Source: CAD feature listing. Evaluate the final solid. Frame: model axes, mm. A direction names the side the tool comes from. Give positions to 0.01 mm unless a question says otherwise; leave off trailing zeros. Order: outer loops, then holes, each group sorted by start corner. A loop starts at its lowest first (then second) coordinate and runs counter-clockwise, first axis right, second up. Notation, with made-up numbers: M -28,-38.5 L -15,-38.5 A28 cw -15,-17.5 Z; hole C 74.25,-3.75 d1. An arc over 180 degrees is marked long. Return JSON: item names as keys, results as strings.
from build123d import *

# Parameters (mm, degrees)
CHAMFER1_SIZE = 0.5


with BuildPart() as part:
    # Sketch1 → Revolve1 (revolve)
    with BuildSketch(Plane.XY, mode=Mode.PRIVATE) as revolve1_sk:
        Polygon((1009, 204.198665167), (1009, 219.898665167), (1006.5, 219.898665167), (1006.5, 222.898665167), (1016.5, 222.898665167), (1016.5, 204.198665167), align=None)
    revolve(revolve1_sk.sketch.rotate(Axis((1016.5, 222.898665167, 0), (0, -1, 0)), 270), axis=Axis((1016.5, 222.898665167, 0), (0, -1, 0)))

    # Chamfer1
    chamfer1_edges = [part.edges().sort_by_distance(p)[0] for p in [
        (1016.5, 222.898665167, -10),
        (1016.5, 219.898665167, -10),
        (1016.5, 204.198665167, -7.5),
    ]]
    chamfer(chamfer1_edges, length=CHAMFER1_SIZE)


solid = part.part
1. Section query D-D (y = 221.25). Return loops of the section in (x, z), then the cut area to 3 significant figures.
Evaluation:
{"outline": "C 1016.5,0 d20", "area": "314 mm^2"}
2. Ray query, probe 1 along Y at (x, z) = (1022.75, -6); probe 2 along X at (y, z) = (212.5, 0.25); probe 3 along Z at (x, y) = (1013, 219.5). Return the intervals inside material, ascending.
Evaluation:
{"probe 1": "y = 219.9 to 222.9", "probe 2": "x = 1009 to 1024", "probe 3": "z = -6.63 to 6.63"}
3. Section query B-B (x = 1016.5). Return loops of the section in (y, z), then the cut area to 3 significant figures.
Evaluation:
{"outline": "M 204.2,-7 L 204.7,-7.5 L 219.9,-7.5 L 219.9,-9.5 L 220.4,-10 L 222.4,-10 L 222.9,-9.5 L 222.9,9.5 L 222.4,10 L 220.4,10 L 219.9,9.5 L 219.9,7.5 L 204.7,7.5 L 204.2,7 Z", "area": "295 mm^2"}
4. First-contact query: pin 1 (1 mm diameter, centred on x = 1020.5, y = 207, fed in from -Z); pin 2 (3 mm diameter, centred on x = 1009, y = 215.5, fed in from +Z); pin 3 (2 mm diameter, centred on x = 1010.5, y = 213, fed in from +Z). Flat tips, straight axial feed; report the tip coordinate or a pass-through.
Evaluation:
{"pin 1": "stops at z = -6.63", "pin 2": "stops at z = 4.5", "pin 3": "stops at z = 5.59"}
5. Section query C-C (y = 214). Return loops of the section in (x, z), then the cut area to 3 significant figures.
Evaluation:
{"outline": "C 1016.5,0 d15", "area": "177 mm^2"}
6. Section query A-A (z = 0). Return loops of the section in (x, y).
Evaluation:
{"outline": "M 1006.5,220.4 L 1007,219.9 L 1009,219.9 L 1009,204.7 L 1009.5,204.2 L 1023.5,204.2 L 1024,204.7 L 1024,219.9 L 1026,219.9 L 1026.5,220.4 L 1026.5,222.4 L 1026,222.9 L 1007,222.9 L 1006.5,222.4 Z"}
7. Set-up query: faces 1 (the face through (1016, 222.899, 0)), 2 (the face through (1008.7, 219.899, -0.7)). Return all of +Z, -Z, +X, -X, +Y, -Y with unobstructed straight access to the full face (end or side cutting, diameter ignored); none if empty.
Evaluation:
{"face 1": "+Z, -Z, +X, -X, +Y", "face 2": "-Y"}
